Here's how the part is built. I have some questions about the finished solid (model axes, mm). Round coordinates to 2 decimals unless told otherwise and drop trailing zeros. Write each loop counter-clockwise with the first axis right and the second up, starting at its lowest first coordinate (ties: lowest second). Pieces come first, ordered by that corner, then holes. Notation, with made-up numbers: (14.25, -27.5) -> (62.25, -27.5) arc R12 cw to (62.25, -15.5) -> close; hole circle Ø3 at (-14, 46). An arc over 180 degrees is marked (long way). Answer as CSV lines item,"result".
```python
from build123d import *
from build123d.topology import SkipClean

# Parameters (mm, degrees)
HUB_RING_SKETCH_R    = 5
HUB_RING_SKETCH_R_2  = 2.5
HUB_RING_10X_5_DEPTH = 4
ARM_ROD_SKETCH_R     = 1.1
ARM_ROD_2_2_DEPTH    = 11.5
ARM_ROOT_SKETCH_R    = 1.1
ARM_ROOT_JOINT_DEPTH = 2.5


with BuildPart() as part:
    # Hub Ring Sketch → Hub Ring Ø10xØ5 (new body)
    with BuildSketch(Plane(origin=(0, 0, 0), x_dir=(1, 0, 0), z_dir=(0, 1, 0))):
        with Locations(Location((0, 0, 0), (0, 0, 270))):
            Circle(HUB_RING_SKETCH_R)
        with Locations(Location((0, 0, 0), (0, 0, 270))):
            Circle(HUB_RING_SKETCH_R_2, mode=Mode.SUBTRACT)
    extrude(amount=HUB_RING_10X_5_DEPTH)



with BuildPart() as body_2:
    # Arm Rod Sketch → Arm Rod Ø2.2 (new body)
    with BuildSketch(Plane(origin=(5, 0, 0), x_dir=(0, 0, -1), z_dir=(1, 0, 0))):
        with Locations((0, 2)):
            Circle(ARM_ROD_SKETCH_R)
    extrude(amount=ARM_ROD_2_2_DEPTH)


with BuildPart() as part_1:
    with SkipClean():  # the faces are left unmerged after this step: merging them gives an invalid solid
        add(part.part)

        add(body_2.part)  # Arm Root Joint merges body 2
        # Arm Root Sketch → Arm Root Joint (add)
        with BuildSketch(Plane(origin=(5, 0, 0), x_dir=(0, 0, -1), z_dir=(1, 0, 0))):
            with Locations((0, 2)):
                Circle(ARM_ROOT_SKETCH_R)
        extrude(amount=-ARM_ROOT_JOINT_DEPTH)


solid = part_1.part
```
1. Suppose I cut it at A-A on x = 2. Please give me the cut outline in (y, z), and give its area (3 significant figures).
Numbers:
outline,"(0, -4.58) -> (4, -4.58) -> (4, -1.5) -> (0, -1.5) -> close; (0, 1.5) -> (4, 1.5) -> (4, 4.58) -> (0, 4.58) -> close"
area,"24.7 mm^2"
2. For pin 1 Ø2 at (x, y) = (14, 2.5) entering from +Z; pin 2 Ø1.5 at (y, z) = (2, -3.5) entering from +X, each with a flat end and sliding along its axis, tell me the tip position at first contact or that it passes through.
Numbers:
pin 1,"stops at z = 1.1"
pin 2,"stops at x = 4.18"
3. Suppose I cut it at B-B on z = -0.25. Please give me the cut outline in (x, y), and give its area (3 significant figures).
Numbers:
outline,"(-4.99, 0) -> (-2.49, 0) -> (-2.49, 4) -> (-4.99, 4) -> close; (2.49, 0) -> (4.99, 0) -> (4.99, 0.93) -> (16.5, 0.93) -> (16.5, 3.07) -> (4.99, 3.07) -> (4.99, 4) -> (2.49, 4) -> close"
area,"44.7 mm^2"
4. Suppose I cut it at C-C on y = 3.7. Please give me the cut outline in (x, z), and give its area (3 significant figures).
Numbers:
outline,"circle Ø10 at (0, 0); hole circle Ø5 at (0, 0)"
area,"58.9 mm^2"
5. Suppose I cut it at D-D on z = 2. Please give me the cut outline in (x, y).
Numbers:
outline,"(-4.58, 0) -> (-1.5, 0) -> (-1.5, 4) -> (-4.58, 4) -> close; (1.5, 0) -> (4.58, 0) -> (4.58, 4) -> (1.5, 4) -> close"
6. If I drill on line 1 (X direction, y = 1.9, z = 0); line 2 (X direction, y = 2.75, z = -2.25); line 3 (Z direction, x = 13.5, y = 2.1), over which ranges is the centre line in solid material (lowest first)?
Numbers:
line 1,"x = -5 to -2.5, 2.5 to 16.5"
line 2,"x = -4.47 to -1.09, 1.09 to 4.47"
line 3,"z = -1.1 to 1.1"
7. If we mould it in two halves opening along X, with no side actions, what happens to faces 1 (the face through (-2, 4, 2)), 2 (the face through (16.5, 2, 0)), 3 (the face through (-2.44, 1.97, -0.54))? For each: released by +X, released by -X, zero draft, split by the parting line, or undercut.
Numbers:
face 1,"zero draft"
face 2,"released by +X"
face 3,"undercut"
